Can you work these out from the model? Positions are in its coordinate system, mm. Face numbers are marked on the shaded views. A direction names the side the tool comes from. Give positions to 0.01 mm unless a question says otherwise; leave off trailing zeros. Order: outer loops, then holes, each group sorted by start corner. A loop starts at its lowest first (then second) coordinate and runs counter-clockwise, first axis right, second up. Notation, with made-up numbers: (-27.75, 57) -> (12.25, 57) arc R25 cw to (12.25, 80) -> close; hole circle Ø4 at (44, 8). An arc over 180 degrees is marked (long way). Answer as CSV lines item,"result".
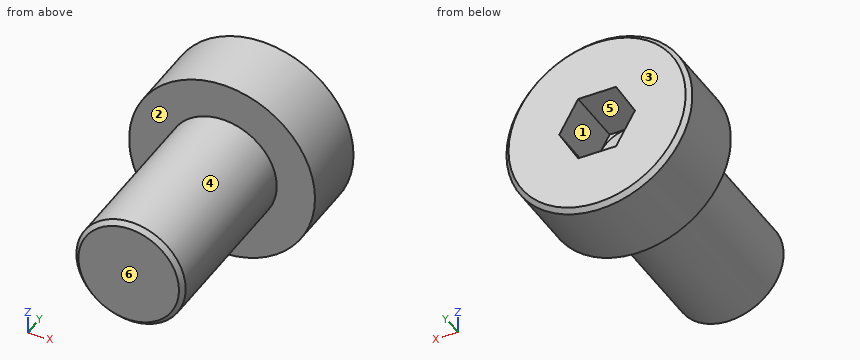
```python
from build123d import *

# Parameters (mm, degrees)
CHAMFER1_SIZE         = 0.2
CUT_EXTRUDE1_DEPTH    = 2.7
BODY_MOVE_COPY1_ANGLE = 180


with BuildPart() as part:
    # Sketch2 → Revolve1 (revolve)
    with BuildSketch(Plane.XY):
        Polygon((1.5, -3.5), (1.5, -0.8), (0, 0.066025404), (0, 8), (2.5, 8), (2.5, 0), (4.25, 0), (4.25, -3.5), align=None)
    revolve(axis=Axis((0, 0.066025404, 0), (0, 1, 0)))

    # Chamfer1
    chamfer1_edges = [part.edges().sort_by_distance(p)[0] for p in [
        (-4.25, -3.5, 0),
        (-2.5, 8, 0),
    ]]
    chamfer(chamfer1_edges, length=CHAMFER1_SIZE)

    # Sketch3 → Cut-Extrude1 (cut)
    with BuildSketch(Plane.XZ.offset(3.5)):
        Polygon((-0.866025404, 1.5), (-1.732050808, 0), (-0.866025404, -1.5), (0.866025404, -1.5), (1.732050808, 0), (0.866025404, 1.5), align=None)
    extrude(amount=-CUT_EXTRUDE1_DEPTH, mode=Mode.SUBTRACT)


with BuildPart() as part_1:
    # Body-Move/Copy1: moved
    add(part.part.rotate(Axis((0, 3.25, 0), (1, 0, 0)), BODY_MOVE_COPY1_ANGLE))


solid = part_1.part
```
Item 1: Imagine slicing it at A-A, the plane y = 5.5. Please give me the cut outline in (x, z), then the cut area to 3 significant figures.
Numbers:
outline,"circle Ø5 at (0, 0)"
area,"19.6 mm²"
Item 2: We'd pull the mould along X, two halves only. Please class the marked faces 4, 5 and 6: released by +X, released by -X, zero draft, split by the parting line, or undercut.
Numbers:
face 4,"split by the parting line"
face 5,"undercut"
face 6,"zero draft"
Item 3: Please list where these lines run through material, in increasing order: line 1 along Y through (x, z) = (3, -0.5); line 2 along X through (y, z) = (8.25, 1); line 3 along Z through (x, y) = (0, -0.25).
Numbers:
line 1,"y = 6.5 to 10"
line 2,"x = -4.13 to -1.15, 1.15 to 4.13"
line 3,"z = -2.5 to 2.5"
Item 4: For the marked faces 1, 2 and 3, which set-ups out of +Z, -Z, +X, -X, +Y, -Y let a thin tool reach every point of the face, with its end or its side?
Numbers:
face 1,"+Y"
face 2,"-Y"
face 3,"+Z, -Z, +X, -X, +Y"
Item 5: For pin 1 (1.5 mm diameter, centred on y = 2, z = 1.5, fed in from -X); pin 2 (2 mm diameter, centred on x = -3, y = 0, fed in from -Z); pin 3 (0.6 mm diameter, centred on x = -0.5, z = -1, fed in from +Y), each with a flat end and sliding along its axis, tell me the tip position at first contact or that it passes through.
Numbers:
pin 1,"stops at x = -2.38"
pin 2,"stops at z = -1.5"
pin 3,"stops at y = 7.25"
